from build123d import *

# Parameters (mm, degrees)
SKETCH1_R           = 12
BOSS_EXTRUDE1_DEPTH = 35
SKETCH2_R           = 3.5
BOSS_EXTRUDE2_DEPTH = 5
SKETCH3_W           = 16
SKETCH3_H           = 25
CUT_EXTRUDE1_DEPTH  = 28
CUT_EXTRUDE2_DEPTH  = 15
CUT_EXTRUDE3_START  = -15
CUT_EXTRUDE3_DEPTH  = 15
SKETCH6_R           = 3
BOSS_EXTRUDE3_DEPTH = 13
SKETCH7_R           = 2.5
BOSS_EXTRUDE4_DEPTH = 12.5
SKETCH8_W           = 9.031547502
SKETCH8_H           = 2.523978301
CUT_EXTRUDE4_DEPTH  = 10


with BuildPart() as part:
    # Sketch1 → Boss-Extrude1 (new body)
    with BuildSketch(Plane.XY):
        Circle(SKETCH1_R)
    extrude(amount=BOSS_EXTRUDE1_DEPTH)

    # Sketch2 → Boss-Extrude2 (add)
    with BuildSketch(Plane(origin=(0, 0, 0), x_dir=(-1, 0, 0), z_dir=(0, 0, -1))):
        Circle(SKETCH2_R)
    extrude(amount=BOSS_EXTRUDE2_DEPTH)

    # Sketch3 → Cut-Extrude1 (cut)
    with BuildSketch(Plane.XY.offset(35)):
        Rectangle(SKETCH3_W, SKETCH3_H)
    extrude(amount=-CUT_EXTRUDE1_DEPTH, mode=Mode.SUBTRACT)

    # Sketch4 → Cut-Extrude2 (cut, symmetric)
    with BuildSketch(Plane(origin=(0, 0, 0), x_dir=(0, 0, -1), z_dir=(1, 0, 0))):
        with BuildLine():
            Line((-28, -2.5), (-35, -2.5))
            Line((-35, -2.5), (-35, 2.5))
            Line((-35, 2.5), (-28, 2.5))
            ThreePointArc((-28, 2.5), (-25.5, 0), (-28, -2.5))
        make_face()
    extrude(amount=CUT_EXTRUDE2_DEPTH, both=True, mode=Mode.SUBTRACT)

    # Sketch5 → Cut-Extrude3 (cut)
    with BuildSketch(Plane.XY.offset(35).offset(CUT_EXTRUDE3_START)):
        with BuildLine():
            Line((11, -4.795831523), (11, 4.795831523))
            ThreePointArc((11, 4.795831523), (12, 0), (11, -4.795831523))
        make_face()
        with BuildLine():
            Line((-11, -4.795831523), (-11, 4.795831523))
            ThreePointArc((-11, 4.795831523), (-12, 0), (-11, -4.795831523))
        make_face()
    extrude(amount=CUT_EXTRUDE3_DEPTH, mode=Mode.SUBTRACT)

    # Sketch6 → Boss-Extrude3 (add)
    with BuildSketch(Plane(origin=(0, 0, -5), x_dir=(-1, 0, 0), z_dir=(0, 0, -1))):
        with Locations(Location((0, 0, 0), (0, 0, 180))):
            Circle(SKETCH6_R)
    extrude(amount=BOSS_EXTRUDE3_DEPTH)

    # Sketch7 → Boss-Extrude4 (add)
    with BuildSketch(Plane(origin=(0, 0, -18), x_dir=(-1, 0, 0), z_dir=(0, 0, -1))):
        Circle(SKETCH7_R)
    extrude(amount=BOSS_EXTRUDE4_DEPTH)

    # Sketch8 → Cut-Extrude4 (cut)
    with BuildSketch(Plane(origin=(0, 0, -30.5), x_dir=(-1, 0, 0), z_dir=(0, 0, -1))):
        with Locations((0, 3.261989151)):
            Rectangle(SKETCH8_W, SKETCH8_H)
    extrude(amount=-CUT_EXTRUDE4_DEPTH, mode=Mode.SUBTRACT)


solid = part.part
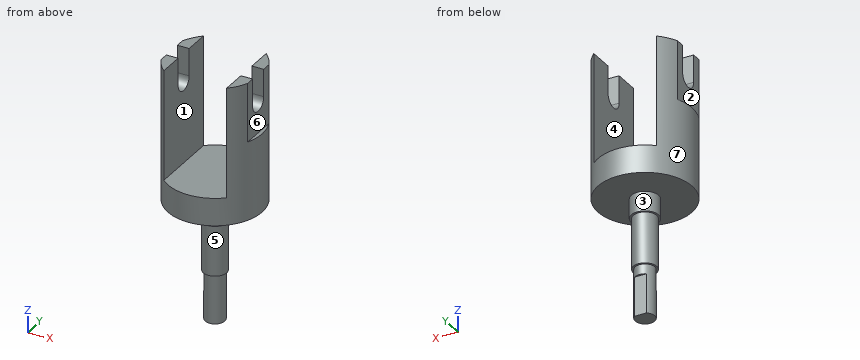
The listing builds one solid part. Answer for the finished solid, in the listing's coordinates (mm). Face numbers are marked on the shaded views. A direction names the side the tool comes from. Round coordinates to 2 decimals unless told otherwise and drop trailing zeros. Loops run counter-clockwise (first coordinate to the right, second up) from the corner with the lowest first, then second, coordinate; pieces in that order, holes last. Notation, with made-up numbers: M 67.25,3 L 104.25,3 A13 cw 104.25,21 Z; hole C 13,3 d4. An arc over 180 degrees is marked long. Write each question's results on one line, items separated by ' | '. Start each with the question number.
1) Straight lines are drawn through the part: probe 1 along Z at (x, y) = (10.75, -3.75); probe 2 along Y at (x, z) = (-0.5, 5); probe 3 along Z at (x, y) = (-2, -9.75). For each, find the intervals that lie inside material, in ascending order.
2) Determine the mould class of the marked faces 1, 2 and 3 for opening direction X: pulls with the +X half, pulls with the -X half, needs draft (parallel to the pull), parting line crosses it, or undercut.
3) Find section A-A on x = 0. Write down the section's boundary in (y, z).
4) Find section C-C on z = -4. Write down the section's boundary in (x, y), plus the area to 3 significant figures.
5) Find section D-D on y = 5.75. Write down the section's boundary in (x, z).
6) Which of the six approach directions +Z, -Z, +X, -X, +Y, -Y give full straight-line access (tool end or side, diameter ignored) to the marked faces 4, 5, 6 and 7?
7) Find section B-B on y = 0. Write down the section's boundary in (x, z), plus the area to 4 significant figures.
8) Each of these flat-tipped pins is pushed along its axis until it touches: pin 1 (1.5 mm diameter, centred on x = -9.5, z = 30, fed in from +Y); pin 2 (1.5 mm diameter, centred on y = -4.5, z = 7, fed in from +X); pin 3 (0.5 mm diameter, centred on x = 11.5, y = -2, fed in from +Z); pin 4 (6 mm diameter, centred on x = 6.5, y = 0.5, fed in from +Z). Where does it stop, or does it pass through?
Final values:
1) probe 1: 0 to 35 | probe 2: -11.99 to 11.99 | probe 3: 0 to 7
2) face 1: undercut | face 2: pulls with the -X half | face 3: parting line crosses it
3) outline: M -12,0 L -3.5,0 L -3.5,-5 L -3,-5 L -3,-18 L -2.5,-18 L -2.5,-30.5 L 2,-30.5 L 2,-20.5 L 2.5,-20.5 L 2.5,-18 L 3,-18 L 3,-5 L 3.5,-5 L 3.5,0 L 12,0 L 12,7 L -12,7 Z
4) outline: C 0,0 d7 | area: 38.5 mm²
5) outline: M -10.53,0 L 10.53,0 L 10.53,35 L 8,35 L 8,7 L -8,7 L -8,35 L -10.53,35 Z
6) face 4: +Z, +Y, -Y | face 5: -Z | face 6: +Z, +X, +Y, -Y | face 7: +Z, -Z
7) outline: M -12,0 L -3.5,0 L -3.5,-5 L -3,-5 L -3,-18 L -2.5,-18 L -2.5,-30.5 L 2.5,-30.5 L 2.5,-18 L 3,-18 L 3,-5 L 3.5,-5 L 3.5,0 L 12,0 L 12,20 L 11,20 L 11,25.5 L 8,25.5 L 8,7 L -8,7 L -8,25.5 L -11,25.5 L -11,20 L -12,20 Z | area: 480.5 mm²
8) pin 1: y = 8.21 | pin 2: x = 11.4 | pin 3: z = 20 | pin 4: z = 35
